Can you work these out from the model? Positions are in its coordinate system, mm. Face numbers are marked on the shaded views. Give positions to 0.01 mm unless a question says otherwise; leave off trailing zeros. Write each loop counter-clockwise with the first axis right and the second up, starting at its lowest first coordinate (ties: lowest second). Pieces come first, ordered by that corner, then holes.
1. If I drill on probe 1 along Y at (x, z) = (9.25, 0); probe 2 along Y at (x, z) = (9.5, 0.75); probe 3 along Z at (x, y) = (-9, 2.75), over which ranges is the centre line in solid material (lowest first)?
2. Suppose I cut it at A-A (x = 4.5). Please give me the cut outline in (y, z), and give its area (3 significant figures).
3. I'm going to push flat-ended pins straight in: pin 1 (1 mm diameter, centred on x = 6.5, y = 2.5, fed in from +Z); pin 2 (1.5 mm diameter, centred on x = 17, z = 7.5, fed in from +Y); pin 3 (10 mm diameter, centred on x = 6.5, z = 6, fed in from +Y); pin 4 (9 mm diameter, centred on y = 0, z = 0, fed in from +X). Where does each tip first touch, or does it pass through?
4. Thinking about a two-plate mould opening in Y: for the marked faces 1, 2, 3 and 4, which applies, pulls with the +Y half, pulls with the -Y half, needs draft (parallel to the pull), parting line crosses it, or undercut?
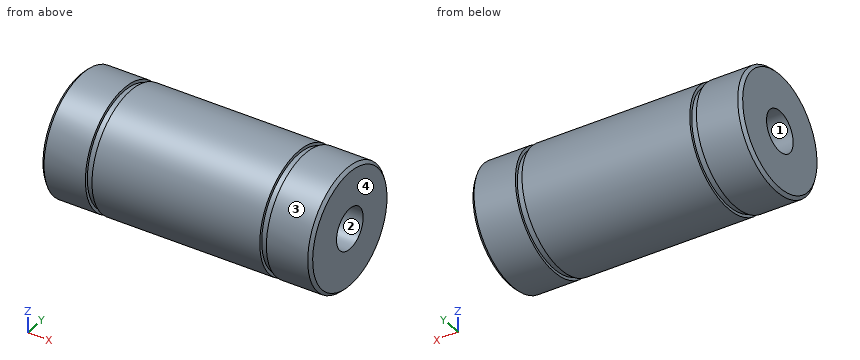
```python
from build123d import *

# Parameters (mm, degrees)
SKETCH_1_R      = 10
EXTRUDE_1_DEPTH = 22.5
CHAMFER_1_SIZE  = 0.5
SKETCH_4_W      = 1.1
SKETCH_4_H      = 0.5


with BuildPart() as part:
    # 草图1 → 凸台-拉伸1 (new, symmetric)
    with BuildSketch(Plane(origin=(0, 0, 0), x_dir=(0, 0, -1), z_dir=(1, 0, 0))):
        with Locations(Location((0, 0, 0), (0, 0, 180))):
            Circle(SKETCH_1_R)
    extrude(amount=EXTRUDE_1_DEPTH, both=True)

    # 草图2 → M8 螺纹孔1 (revolve, cut)
    with BuildSketch(Plane(origin=(22.5, 0, 0), x_dir=(0, 0, -1), z_dir=(0, 1, 0))):
        Polygon((0, 0), (0, 21.792926105), (3.4, 19.75), (3.4, 0), align=None)
    hole_wizard_m8_1 = revolve(axis=Axis((28.85, 0, 0), (-1, 0, 0)), mode=Mode.SUBTRACT)

    # 镜向1: M8 螺纹孔1 across plane
    add(hole_wizard_m8_1.mirror(Plane(origin=(0, 0, 0), x_dir=(0, 0, 1), z_dir=(1, 0, 0))), mode=Mode.SUBTRACT)

    # 倒角1
    chamfer_1_edges = [part.edges().sort_by_distance(p)[0] for p in [
        (-22.5, 0, -10),
        (22.5, 0, -10),
    ]]
    chamfer(chamfer_1_edges, length=CHAMFER_1_SIZE)

    # 草图4 → 切除-旋转1 (revolve, cut)
    with BuildSketch(Plane.XY, mode=Mode.PRIVATE) as cut_revolve_1_sk:
        with Locations((-14.55, 9.75)):
            Rectangle(SKETCH_4_W, SKETCH_4_H)
    cut_revolve_1 = revolve(cut_revolve_1_sk.sketch.rotate(Axis((0, 0, 0), (1, 0, 0)), 90), axis=Axis((0, 0, 0), (1, 0, 0)), mode=Mode.SUBTRACT)

    # 镜向2: 切除-旋转1 across plane
    add(cut_revolve_1.mirror(Plane(origin=(0, 0, 0), x_dir=(0, 0, 1), z_dir=(1, 0, 0))), mode=Mode.SUBTRACT)


solid = part.part
```
Checks:
1. probe 1: y = -10 to -3.4, 3.4 to 10
1. probe 2: y = -9.97 to -3.32, 3.32 to 9.97
1. probe 3: z = -9.61 to -2, 2 to 9.61
2. outline: circle Ø20 at (0, 0); hole circle Ø6.8 at (0, 0)
2. area: 278 mm2
3. pin 1: stops at z = 9.8
3. pin 2: stops at y = 7.38
3. pin 3: stops at y = 9.95
3. pin 4: stops at x = 22.5
4. face 1: undercut
4. face 2: undercut
4. face 3: parting line crosses it
4. face 4: needs draft
